Part print with two shaded views. Sizes in mm from the minimum x, y, z corner. Round coordinates to 2 decimals unless told otherwise and drop trailing zeros. Order: outer loops, then holes, each group sorted by start corner. A loop starts at its lowest first (then second) coordinate and runs counter-clockwise, first axis right, second up. Notation, with made-up numbers: M -17,-35.75 L -3,-35.75 A24 ccw -3,-4.75 Z; hole C 59.25,89.5 d1. An arc over 180 degrees is marked long. Put each result on its own line as item: value.
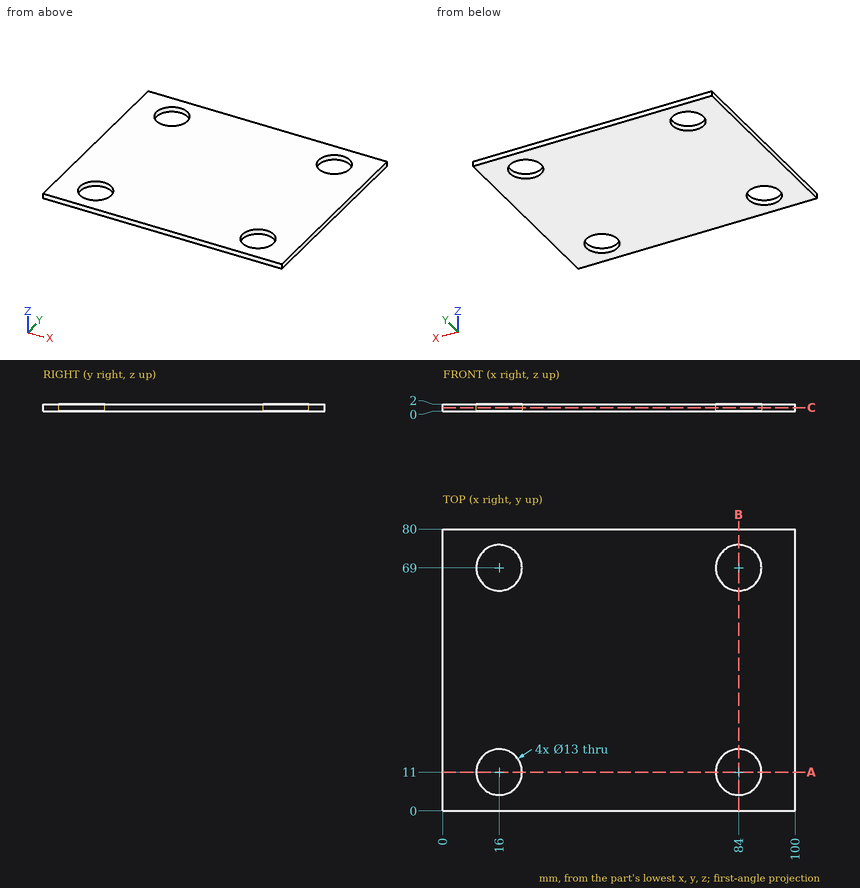
Item 1: Band-saw the part on C-C on z = 0.95. Give the cut face in (x, y), and give its area (3 significant figures).
Answers below:
outline: M 0,0 L 100,0 L 100,80 L 0,80 Z; hole C 16,11 d13; hole C 16,69 d13; hole C 84,11 d13; hole C 84,69 d13
area: 7,470 mm²
Item 2: Pin check, flat tip, straight feed: P1, Ø11.5, axis at x = 16, y = 69, coming from the +Z side. Stop position of the tip, or through.
Answers below:
P1: through
Item 3: Probe line 1 along X through (y, z) = (68.5, 1.05); line 2 along Y through (x, z) = (16, 0.85); line 3 along X through (y, z) = (73, 1.15). List the from-to ranges inside material, lowest first. Write a range as [from, to].
Answers below:
line 1: [0, 9.52], [22.48, 77.52], [90.48, 100]
line 2: [0, 4.5], [17.5, 62.5], [75.5, 80]
line 3: [0, 10.88], [21.12, 78.88], [89.12, 100]
Item 4: Band-saw the part on B-B on x = 84. Give the cut face in (y, z).
Answers below:
outline: M 0,0 L 4.5,0 L 4.5,2 L 0,2 Z; M 17.5,0 L 62.5,0 L 62.5,2 L 17.5,2 Z; M 75.5,0 L 80,0 L 80,2 L 75.5,2 Z
Item 5: Band-saw the part on A-A on y = 11. Give the cut face in (x, z), and give its area (3 significant figures).
Answers below:
outline: M 0,0 L 9.5,0 L 9.5,2 L 0,2 Z; M 22.5,0 L 77.5,0 L 77.5,2 L 22.5,2 Z; M 90.5,0 L 100,0 L 100,2 L 90.5,2 Z
area: 148 mm²
